Could you check a few things on this model? Use its own coordinates, in mm. Give positions to 0.01 mm unless a question says otherwise; leave off trailing zeros. Loops run counter-clockwise (first coordinate to the right, second up) from the corner with the lowest first, then second, coordinate; pieces in that order, holes last. Notation, with made-up numbers: M 65,-24 L 76,-24 A24 ccw 76,-2 Z; hole C 65.5,34.5 d3. An arc over 180 degrees is marked long. Answer in a Markdown table with one row per item. Add a question column.
```python
from build123d import *

# Parameters (mm, degrees)
SKETCH1_W                    = 140
SKETCH1_H                    = 110
BOSS_EXTRUDE1_DEPTH          = 14
FILLET1_R                    = 5
M12_TAPPED_HOLE1_D           = 10.2
M12_TAPPED_HOLE1_DEPTH       = 32.75
M12_TAPPED_HOLE1_CSINK_D     = 12.05
M12_TAPPED_HOLE1_CSINK_ANGLE = 90
M12_TAPPED_HOLE1_TIP         = 3.064389157


with BuildPart() as part:
    # Sketch1 → Boss-Extrude1 (new body)
    with BuildSketch(Plane(origin=(0, 0, 0), x_dir=(0, 0, -1), z_dir=(1, 0, 0))):
        Rectangle(SKETCH1_W, SKETCH1_H)
    extrude(amount=BOSS_EXTRUDE1_DEPTH)

    # Fillet1
    fillet1_edges = [part.edges().sort_by_distance(p)[0] for p in [
        (7, -55, -70),
        (7, -55, 70),
        (7, 55, 70),
        (7, 55, -70),
    ]]
    fillet(fillet1_edges, radius=FILLET1_R)

    # M12 Tapped Hole1
    with Locations(Plane.ZY):
        with Locations((-52.5, 34.756569307), (52.499717816, 35), (52.5, -35), (-52.5, -35.243430693)):
            CounterSinkHole(M12_TAPPED_HOLE1_D / 2, M12_TAPPED_HOLE1_CSINK_D / 2, depth=M12_TAPPED_HOLE1_DEPTH, counter_sink_angle=M12_TAPPED_HOLE1_CSINK_ANGLE)
            with Locations((0, 0, -(M12_TAPPED_HOLE1_DEPTH + M12_TAPPED_HOLE1_TIP / 2))):  # 118° drill point
                Cone(0, M12_TAPPED_HOLE1_D / 2, M12_TAPPED_HOLE1_TIP, mode=Mode.SUBTRACT)


solid = part.part
```
Item 1: If we mould it in two halves opening along Y, with no side actions, what happens to faces 1 (the face through (7, 53, 69)), 2 (the face through (7.55, -38.1, 56.55)), 3 (the face through (7, -1, -70))? For each: +Y half, -Y half, draft (parallel to the pull), parting line (faces both ways), or undercut.
Item 2: Suppose I cut it at A-A (x = 11.75). List the corners of the cut face in (y, z) for me.
Item 3: I need wall thicknesses on L1, parallel to Z at x = 8.75, y = 34.5; L2, parallel to Y at x = 7, z = -52.5; L3, parallel to Y at x = 11, z = 52.5. Which ranges of each line are inside material? Lowest first, please.
Item 4: Suppose I cut it at B-B (z = 52.5). Give the number of separate pieces and of enclosed holes in the cut face, then the cut area to 3 significant figures.
Values found:
| question | item | result |
|---|---|---|
| 1 | face 1 | +Y half |
| 1 | face 2 | undercut |
| 1 | face 3 | draft |
| 2 | outline | M -55,-65 A5 ccw -50,-70 L 50,-70 A5 ccw 55,-65 L 55,65 A5 ccw 50,70 L -50,70 A5 ccw -55,65 Z; hole C -35.24,-52.5 d10.2; hole C -35,52.5 d10.2; hole C 34.76,-52.5 d10.2; hole C 35,52.5 d10.2 |
| 3 | L1 | -70 to -57.59, -47.41 to 47.42, 57.58 to 70 |
| 3 | L2 | -55 to -40.34, -30.14 to 29.66, 39.86 to 55 |
| 3 | L3 | -55 to -40.1, -29.9 to 29.9, 40.1 to 55 |
| 4 | separate pieces | 3 |
| 4 | enclosed holes | 0 |
| 4 | area | 1,250 mm² |
